Here's how the part is built. I have some questions about the finished solid (model axes, mm). Coordinates: 2 decimals unless noted, no trailing zeros. Write each loop counter-clockwise with the first axis right and the second up, starting at its lowest first coordinate (ties: lowest second). Pieces come first, ordered by that corner, then holes.
(1) Please list where these lines run through material, in increasing order: probe 1 along Y at (x, z) = (25, 16); probe 2 along Y at (x, z) = (31, 8.5).
(2) For pin 1 Ø14 at (x, y) = (125, 25) entering from -Z, with a flat end and sliding along its axis, tell me the tip position at first contact or that it passes through.
(3) Imagine slicing it at A-A, the plane y = 25. List the corners of the cut face in (x, z) for me, plus the area to 3 significant figures.
(4) Imagine slicing it at C-C, the plane x = 125. List the corners of the cut face in (y, z) for me, plus the area to 3 significant figures.
(5) Thinking about a two-plate mould opening in X: for faces 1 (the flat face through (150, 99, 15)), 2 (the flat face through (74, 101, 30)), 3 (the cylindrical face through (133.74, 25.38, 14.79)), which applies, released by +X, released by -X, zero draft, split by the parting line, or undercut?
(6) Imagine slicing it at B-B, the plane z = 22. List the corners of the cut face in (x, y) for me, plus the area to 3 significant figures.
```python
from build123d import *

# Parameters (mm, degrees)
SKETCH1_W            = 150
SKETCH1_H            = 200
BOSS_EXTRUDE1_DEPTH  = 30
M20_THREADED_HOLE1_D = 17.5


with BuildPart() as part:
    # Sketch1 → Boss-Extrude1 (new body)
    with BuildSketch(Plane.XY):
        with Locations((75, 100)):
            Rectangle(SKETCH1_W, SKETCH1_H)
    extrude(amount=BOSS_EXTRUDE1_DEPTH)

    # M20 Threaded hole1 (through all)
    with Locations(Plane(origin=(25, 175, 30), x_dir=(1, 0, 0), z_dir=(0, 0, 1))):
        with Locations((0, 0), (100, 0), (0, -150), (100, -150)):
            Hole(M20_THREADED_HOLE1_D / 2)


solid = part.part
```
Recorded:
1. probe 1: y = 0 to 16.25, 33.75 to 166.25, 183.75 to 200
1. probe 2: y = 0 to 18.63, 31.37 to 168.63, 181.37 to 200
2. pin 1: passes through
3. outline: (0, 0) - (16.25, 0) - (16.25, 30) - (0, 30) - close; (33.75, 0) - (116.25, 0) - (116.25, 30) - (33.75, 30) - close; (133.75, 0) - (150, 0) - (150, 30) - (133.75, 30) - close
3. area: 3,450 mm2
4. outline: (0, 0) - (16.25, 0) - (16.25, 30) - (0, 30) - close; (33.75, 0) - (166.25, 0) - (166.25, 30) - (33.75, 30) - close; (183.75, 0) - (200, 0) - (200, 30) - (183.75, 30) - close
4. area: 4,950 mm2
5. face 1: released by +X
5. face 2: zero draft
5. face 3: undercut
6. outline: (0, 0) - (150, 0) - (150, 200) - (0, 200) - close; hole circle Ø17.5 at (25, 25); hole circle Ø17.5 at (25, 175); hole circle Ø17.5 at (125, 25); hole circle Ø17.5 at (125, 175)
6. area: 29,000 mm2
